Input: dimensioned drawing with shaded views. Units: mm. Origin: part minimum x, y, z. Round coordinates to 2 decimals unless told otherwise and drop trailing zeros. Loops run counter-clockwise (first coordinate to the right, second up) from the corner with the lowest first, then second, coordinate; pieces in that order, holes last. Notation, with made-up numbers: M 9,-8 L 21,-8 A33 cw 21,25 Z; hole C -22,-8.75 d6. An arc over 180 degrees is marked long. Write each question's results on one line, items separated by ' | '. Start each with the question number.
1. Contact query for flat-ended pins moving along their axis: pin 1 Ø1.5 at (x, y) = (105.5, 9) entering from -Z; pin 2 Ø14.5 at (x, z) = (112.12, 291.56) entering from +Y; pin 3 Ø4 at (y, z) = (3.5, 251) entering from +X; pin 4 Ø2 at (x, y) = (136.5, 3) entering from +Z. Output: stop coordinate, or through.
2. Section A-A on x = 160. Output: boundary loops of the cut face in (y, z).
3. Section B-B on z = 160. Output: boundary loops of the cut face in (x, y).
4. Section D-D on y = 7.25. Give the number of separate pieces and of enclosed holes in the cut face, and give its area (3 significant figures).
5. Ray query, line 1 (Z direction, x = 159.5, y = 3) (1 decimal); line 2 (Z direction, x = 115, y = 5) (1 decimal); line 3 (X direction, y = 6, z = 230) (1 decimal). Return the intervals inside material, ascending.
6. Section C-C on z = 230. Output: boundary loops of the cut face in (x, y) (1 decimal).
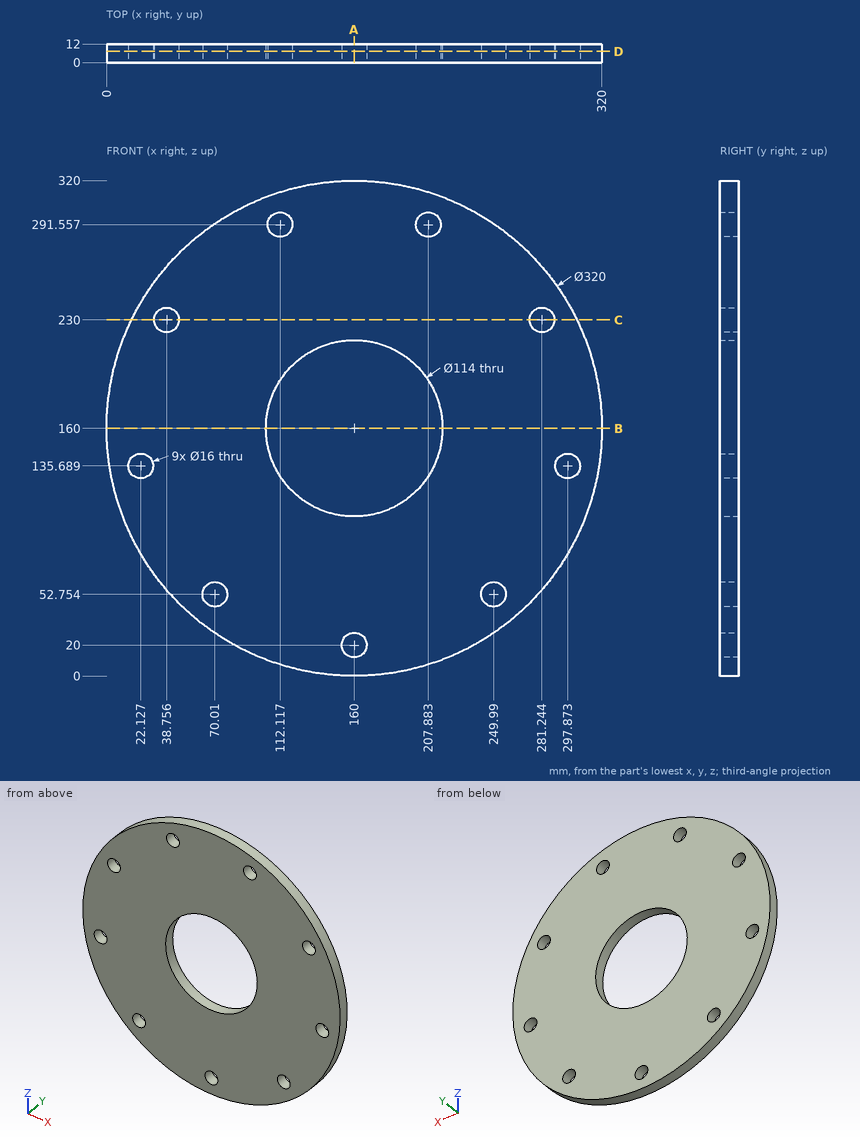
Taken from the geometry:
1) pin 1: z = 9.3 | pin 2: through | pin 3: x = 292.96 | pin 4: z = 318.41
2) outline: M 0,0 L 12,0 L 12,12 L 0,12 Z; M 0,28 L 12,28 L 12,103 L 0,103 Z; M 0,217 L 12,217 L 12,320 L 0,320 Z
3) outline: M 0,0 L 103,0 L 103,12 L 0,12 Z; M 217,0 L 320,0 L 320,12 L 217,12 Z
4) separate pieces: 1 | enclosed holes: 10 | area: 68,400 mm^2
5) line 1: 0 to 12, 28 to 103, 217 to 320 | line 2: 6.5 to 125, 195 to 284.1, 299 to 313.5 | line 3: 16.1 to 30.8, 46.8 to 273.2, 289.2 to 303.9
6) outline: M 16.1,0 L 30.8,0 L 30.8,12 L 16.1,12 Z; M 46.8,0 L 273.2,0 L 273.2,12 L 46.8,12 Z; M 289.2,0 L 303.9,0 L 303.9,12 L 289.2,12 Z
